```python
from build123d import *


with BuildPart() as part:
    # 草图1 → 旋转1 (revolve)
    with BuildSketch(Plane.XY, mode=Mode.PRIVATE) as revolve_1_sk:
        Polygon((7.5, 0), (7.5, -9), (9.5, -9), (9.5, -8), (13.5, -8), (13.5, -9), (16, -9), (16, 0), (13.5, 0), (13.5, -0.807209449), (9.5, -0.807209449), (9.5, 0), align=None)
    revolve(revolve_1_sk.sketch.rotate(Axis((0, 13.438321286, 0), (0, -1, 0)), 90), axis=Axis((0, 13.438321286, 0), (0, -1, 0)))


solid = part.part
```
Part model, mm, in its own coordinate system. A direction names the side the tool comes from. Coordinates: 2 decimals unless noted, no trailing zeros. Loops run counter-clockwise (first coordinate to the right, second up) from the corner with the lowest first, then second, coordinate; pieces in that order, holes last. Notation, with made-up numbers: (10, -27.75) - (44, -27.75) arc R19 ccw to (44, -20.75) - close; hole circle Ø1 at (77.5, 83.25). An arc over 180 degrees is marked (long way). Write item = value, one per line. Start each with the question number.
Item 1: Cut at C-C, the plane y = -8.5. Give the cut face in (x, z), and give its area (3 significant figures).
Item 2: Cut at A-A, the plane x = 0. Give the cut face in (y, z), and give its area (3 significant figures).
Item 3: Cut at D-D, the plane x = -11. Give the cut face in (y, z), and give its area (3 significant figures).
Item 4: Wall check: L1, parallel to X at y = -0.4, z = 0; L2, parallel to X at y = -0.25, z = -1.5; L3, parallel to Z at x = 5, y = -5.75. Give the ranges that are in metal, low to high. Write a range as from..to.
Item 5: Flat gauge pins, fed straight in: pin 1 Ø5 at (y, z) = (-6, 3.5) entering from -X; pin 2 Ø1.5 at (y, z) = (-7.5, -6) entering from +X; pin 3 Ø4 at (x, y) = (-3.5, -7) entering from -Z. Where does each tip first touch, or does it go through?
Item 6: Cut at B-B, the plane z = 0. Give the cut face in (x, y).
Item 7: 3-axis set-ups, long thin cutter, end or side, ignore diameter. For faces 1 (the cylindrical face through (-6.324, -4.563, 4.032)), 2 (the flat face through (-9.2, -0.807, -3.2)), 3 (the cylindrical face through (9.274, -8.493, -2.059)): which of +Z, -Z, +X, -X, +Y, -Y reach the whole face in a straight line?
The answers:
q1.outline = circle Ø32 at (0, 0); circle Ø19 at (0, 0); hole circle Ø27 at (0, 0); hole circle Ø15 at (0, 0)
q1.area = 339 mm2
q2.outline = (-9, -16) - (0, -16) - (0, -13.5) - (-0.81, -13.5) - (-0.81, -9.5) - (0, -9.5) - (0, -7.5) - (-9, -7.5) - (-9, -9.5) - (-8, -9.5) - (-8, -13.5) - (-9, -13.5) - close; (-9, 7.5) - (0, 7.5) - (0, 9.5) - (-0.81, 9.5) - (-0.81, 13.5) - (0, 13.5) - (0, 16) - (-9, 16) - (-9, 13.5) - (-8, 13.5) - (-8, 9.5) - (-9, 9.5) - close
q2.area = 139 mm2
q3.outline = (-9, -11.62) - (0, -11.62) - (0, -7.83) - (-0.81, -7.83) - (-0.81, 7.83) - (0, 7.83) - (0, 11.62) - (-9, 11.62) - (-9, 7.83) - (-8, 7.83) - (-8, -7.83) - (-9, -7.83) - close
q3.area = 181 mm2
q4.L1 = -16..-13.5, -9.5..-7.5, 7.5..9.5, 13.5..16
q4.L2 = -15.93..-13.42, -9.38..-7.35, 7.35..9.38, 13.42..15.93
q4.L3 = -15.2..-5.59, 5.59..15.2
q5.pin_1 = -15.97
q5.pin_2 = 15.11
q5.pin_3 = -15.93
q6.outline = (-16, -9) - (-13.5, -9) - (-13.5, -8) - (-9.5, -8) - (-9.5, -9) - (-7.5, -9) - (-7.5, 0) - (-9.5, 0) - (-9.5, -0.81) - (-13.5, -0.81) - (-13.5, 0) - (-16, 0) - close; (7.5, -9) - (9.5, -9) - (9.5, -8) - (13.5, -8) - (13.5, -9) - (16, -9) - (16, 0) - (13.5, 0) - (13.5, -0.81) - (9.5, -0.81) - (9.5, 0) - (7.5, 0) - close
q7.face_1 = +Y, -Y
q7.face_2 = +Y
q7.face_3 = -Y
